Can you work these out from the model? Positions are in its coordinate system, mm. A direction names the side the tool comes from. Round coordinates to 2 decimals unless told otherwise and drop trailing zeros. Write each loop counter-clockwise with the first axis right and the second up, starting at its lowest first coordinate (ties: lowest second). Pieces come first, ordered by that corner, then holes.
Q1. For faces 1 (the flat face through (-242.75, 67, -173)), 2 (the flat face through (-3, 0, 0)), which set-ups out of +Z, -Z, +X, -X, +Y, -Y let a thin tool reach every point of the face, with its end or its side?
Q2. If we section it at A-A (y = -13): Please give me the cut outline in (x, z).
Q3. If we section it at D-D (x = -11): Please give me the cut outline in (y, z).
Q4. Please list where these lines run through material, in increasing order: line 1 along X through (y, z) = (-62, 0.9); line 2 along Y through (x, z) = (-239, -346); line 3 along Z through (x, y) = (190.5, 33).
Q5. If we section it at B-B (x = 121): Please give me the cut outline in (y, z).
Q6. I'm going to push flat-ended pins straight in: pin 1 Ø4.5 at (x, y) = (239, -62) entering from +Z; pin 2 Ø4.5 at (x, y) = (100, -62) entering from -Z; pin 3 Ø2 at (x, z) = (52.5, -250.5) entering from -Y. Where does each tip first touch, or does it pass through?
Q7. If we section it at C-C (z = -81.5): Please give me the cut outline in (x, y).
from build123d import *

# Parameters (mm, degrees)
SKETCH1_W                                       = 485.5
SKETCH1_H                                       = 132
BOSS_EXTRUDE1_DEPTH                             = 3
SKETCH2_W                                       = 485.5
SKETCH2_H                                       = 351
BOSS_EXTRUDE2_DEPTH                             = 3
SKETCH3_W                                       = 485.5
SKETCH3_H                                       = 3
BOSS_EXTRUDE3_DEPTH                             = 132
FILLET1_R                                       = 1
FILLET2_R                                       = 6
SKETCH4_W                                       = 40
SKETCH4_H                                       = 10.5
CUT_EXTRUDE1_DEPTH                              = 4.5
SKETCH5_W                                       = 40
SKETCH5_H                                       = 10.5
CUT_EXTRUDE2_DEPTH                              = 4.5
CROSS_RECESS_WOOD_SCREW_HOLE_TYPE_1_D           = 3.4
CROSS_RECESS_WOOD_SCREW_HOLE_TYPE_1_CSINK_D     = 6.6
CROSS_RECESS_WOOD_SCREW_HOLE_TYPE_1_CSINK_ANGLE = 90
CROSS_RECESS_WOOD_SCREW_HOLE_TYPE_2_D           = 3.4
CROSS_RECESS_WOOD_SCREW_HOLE_TYPE_2_DEPTH       = 6.5
CROSS_RECESS_WOOD_SCREW_HOLE_TYPE_2_CSINK_D     = 6.6
CROSS_RECESS_WOOD_SCREW_HOLE_TYPE_2_CSINK_ANGLE = 90
CROSS_RECESS_WOOD_SCREW_HOLE_TYPE_2_TIP         = 1.021463052
CROSS_RECESS_WOOD_SCREW_HOLE_TYPE_3_D           = 3.4
CROSS_RECESS_WOOD_SCREW_HOLE_TYPE_3_DEPTH       = 6.5
CROSS_RECESS_WOOD_SCREW_HOLE_TYPE_3_CSINK_D     = 6.6
CROSS_RECESS_WOOD_SCREW_HOLE_TYPE_3_CSINK_ANGLE = 90
CROSS_RECESS_WOOD_SCREW_HOLE_TYPE_3_TIP         = 1.021463052


with BuildPart() as part:
    # Sketch1 → Boss-Extrude1 (new body)
    with BuildSketch(Plane.XY):
        Rectangle(SKETCH1_W, SKETCH1_H)
    extrude(amount=BOSS_EXTRUDE1_DEPTH)

    # Sketch2 → Boss-Extrude2 (add)
    with BuildSketch(Plane(origin=(0, 66, 0), x_dir=(1, 0, 0), z_dir=(0, 1, 0))):
        with Locations((0, 172.5)):
            Rectangle(SKETCH2_W, SKETCH2_H)
    extrude(amount=BOSS_EXTRUDE2_DEPTH)

    # Sketch3 → Boss-Extrude3 (add)
    with BuildSketch(Plane.XZ.offset(-66)):
        with Locations((0, -346.5)):
            Rectangle(SKETCH3_W, SKETCH3_H)
    extrude(amount=BOSS_EXTRUDE3_DEPTH)

    # Fillet1
    fillet1_edges = [part.edges().sort_by_distance(p)[0] for p in [
        (0, 66, -345),
        (0, 66, 0),
    ]]
    fillet(fillet1_edges, radius=FILLET1_R)

    # Fillet2
    fillet2_edges = [part.edges().sort_by_distance(p)[0] for p in [
        (0, 69, 3),
        (0, 69, -348),
    ]]
    fillet(fillet2_edges, radius=FILLET2_R)

    # Sketch4 → Cut-Extrude1 (cut)
    with BuildSketch(Plane.XY.offset(3)):
        with Locations((0, -60.75)):
            Rectangle(SKETCH4_W, SKETCH4_H)
    extrude(amount=-CUT_EXTRUDE1_DEPTH, mode=Mode.SUBTRACT)

    # Sketch5 → Cut-Extrude2 (cut)
    with BuildSketch(Plane(origin=(0, 0, -348), x_dir=(-1, 0, 0), z_dir=(0, 0, -1))):
        with Locations((150, -60.75)):
            Rectangle(SKETCH5_W, SKETCH5_H)
        with Locations((-150, -60.75)):
            Rectangle(SKETCH5_W, SKETCH5_H)
    extrude(amount=-CUT_EXTRUDE2_DEPTH, mode=Mode.SUBTRACT)

    # Cross recess wood screw hole type 1 (through all)
    with Locations(Plane(origin=(0, 69, 0), x_dir=(1, 0, 0), z_dir=(0, 1, 0))):
        with Locations((239, 332), (239, 172.5), (239, 13), (-239, 332), (-239, 172.5), (-239, 13)):
            CounterSinkHole(CROSS_RECESS_WOOD_SCREW_HOLE_TYPE_1_D / 2, CROSS_RECESS_WOOD_SCREW_HOLE_TYPE_1_CSINK_D / 2, counter_sink_angle=CROSS_RECESS_WOOD_SCREW_HOLE_TYPE_1_CSINK_ANGLE)

    # Cross recess wood screw hole type 2
    with Locations(Plane.XY.offset(3)):
        with Locations((-239, 53), (-239, -62), (-100, -62), (100, -62), (239, 53), (239, -62)):
            CounterSinkHole(CROSS_RECESS_WOOD_SCREW_HOLE_TYPE_2_D / 2, CROSS_RECESS_WOOD_SCREW_HOLE_TYPE_2_CSINK_D / 2, depth=CROSS_RECESS_WOOD_SCREW_HOLE_TYPE_2_DEPTH, counter_sink_angle=CROSS_RECESS_WOOD_SCREW_HOLE_TYPE_2_CSINK_ANGLE)
            with Locations((0, 0, -(CROSS_RECESS_WOOD_SCREW_HOLE_TYPE_2_DEPTH + CROSS_RECESS_WOOD_SCREW_HOLE_TYPE_2_TIP / 2))):  # 118° drill point
                Cone(0, CROSS_RECESS_WOOD_SCREW_HOLE_TYPE_2_D / 2, CROSS_RECESS_WOOD_SCREW_HOLE_TYPE_2_TIP, mode=Mode.SUBTRACT)

    # Cross recess wood screw hole type 3
    with Locations(Plane(origin=(0, 0, -348), x_dir=(-1, 0, 0), z_dir=(0, 0, -1))):
        with Locations((239, 53), (239, -62), (100, -62), (-100, -62), (-239, -62), (-239, 53)):
            CounterSinkHole(CROSS_RECESS_WOOD_SCREW_HOLE_TYPE_3_D / 2, CROSS_RECESS_WOOD_SCREW_HOLE_TYPE_3_CSINK_D / 2, depth=CROSS_RECESS_WOOD_SCREW_HOLE_TYPE_3_DEPTH, counter_sink_angle=CROSS_RECESS_WOOD_SCREW_HOLE_TYPE_3_CSINK_ANGLE)
            with Locations((0, 0, -(CROSS_RECESS_WOOD_SCREW_HOLE_TYPE_3_DEPTH + CROSS_RECESS_WOOD_SCREW_HOLE_TYPE_3_TIP / 2))):  # 118° drill point
                Cone(0, CROSS_RECESS_WOOD_SCREW_HOLE_TYPE_3_D / 2, CROSS_RECESS_WOOD_SCREW_HOLE_TYPE_3_TIP, mode=Mode.SUBTRACT)


solid = part.part
A:
1. face 1: +Z, -Z, -X, +Y, -Y
1. face 2: +X, -X, -Y
2. outline: (-242.75, -348) - (242.75, -348) - (242.75, -345) - (-242.75, -345) - close; (-242.75, 0) - (242.75, 0) - (242.75, 3) - (-242.75, 3) - close
3. outline: (-66, -348) - (63, -348) arc R6 ccw to (69, -342) - (69, -3) arc R6 ccw to (63, 3) - (-55.5, 3) - (-55.5, 0) - (65, 0) arc R1 cw to (66, -1) - (66, -344) arc R1 cw to (65, -345) - (-66, -345) - close
4. line 1: x = -242.75 to -240.7, -237.3 to -101.7, -98.3 to -20, 20 to 98.3, 101.7 to 237.3, 240.7 to 242.75
4. line 2: y = -66 to -63.7, -60.3 to 51.3, 54.7 to 67.47
4. line 3: z = -348 to -345, 0 to 3
5. outline: (-66, -348) - (63, -348) arc R6 ccw to (69, -342) - (69, -3) arc R6 ccw to (63, 3) - (-66, 3) - (-66, 0) - (65, 0) arc R1 cw to (66, -1) - (66, -344) arc R1 cw to (65, -345) - (-66, -345) - close
6. pin 1: stops at z = 1.95
6. pin 2: stops at z = -346.95
6. pin 3: stops at y = 66
7. outline: (-242.75, 66) - (242.75, 66) - (242.75, 69) - (-242.75, 69) - close
